Input: dimensioned drawing with shaded views. Units: mm. Origin: part minimum x, y, z. Coordinates: 2 decimals unless noted, no trailing zeros. Order: outer loops, then holes, each group sorted by start corner. A loop starts at its lowest first (then second) coordinate and runs counter-clockwise, first axis right, second up. Notation, with made-up numbers: (66, 78.5) -> (73, 78.5) arc R31 ccw to (73, 106.5) -> close; hole circle Ø9 at (67.25, 23.25). An arc over 180 degrees is marked (long way). Answer as CSV lines item,"result".
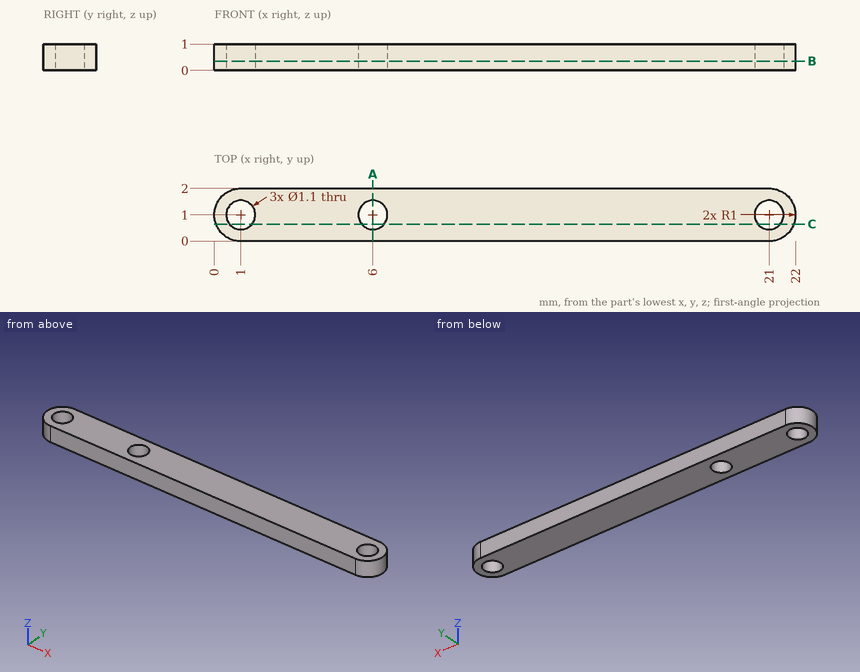
1. Cut plane C-C (y = 0.65). Return the cut outline in (x, z), plus the area to 3 significant figures.
Findings:
outline,"(0.06, 0) -> (0.58, 0) -> (0.58, 1) -> (0.06, 1) -> close; (1.42, 0) -> (5.58, 0) -> (5.58, 1) -> (1.42, 1) -> close; (6.42, 0) -> (20.58, 0) -> (20.58, 1) -> (6.42, 1) -> close; (21.42, 0) -> (21.94, 0) -> (21.94, 1) -> (21.42, 1) -> close"
area,"19.3 mm2"
2. Ray query, line 1 along Y through (x, z) = (6, 0.5); line 2 along X through (y, z) = (0.95, 0.35); line 3 along X through (y, z) = (0.65, 0.15). Return the intervals inside material, ascending.
Findings:
line 1,"y = 0 to 0.45, 1.55 to 2"
line 2,"x = 0 to 0.45, 1.55 to 5.45, 6.55 to 20.45, 21.55 to 22"
line 3,"x = 0.06 to 0.58, 1.42 to 5.58, 6.42 to 20.58, 21.42 to 21.94"
3. Cut plane B-B (z = 0.35). Return the cut outline in (x, y).
Findings:
outline,"(1, 0) -> (21, 0) arc R1 ccw to (21, 2) -> (1, 2) arc R1 ccw to start; hole circle Ø1.1 at (1, 1); hole circle Ø1.1 at (6, 1); hole circle Ø1.1 at (21, 1)"
4. Cut plane A-A (x = 6). Return the cut outline in (y, z), plus the area to 3 significant figures.
Findings:
outline,"(0, 0) -> (0.45, 0) -> (0.45, 1) -> (0, 1) -> close; (1.55, 0) -> (2, 0) -> (2, 1) -> (1.55, 1) -> close"
area,"0.900 mm2"
